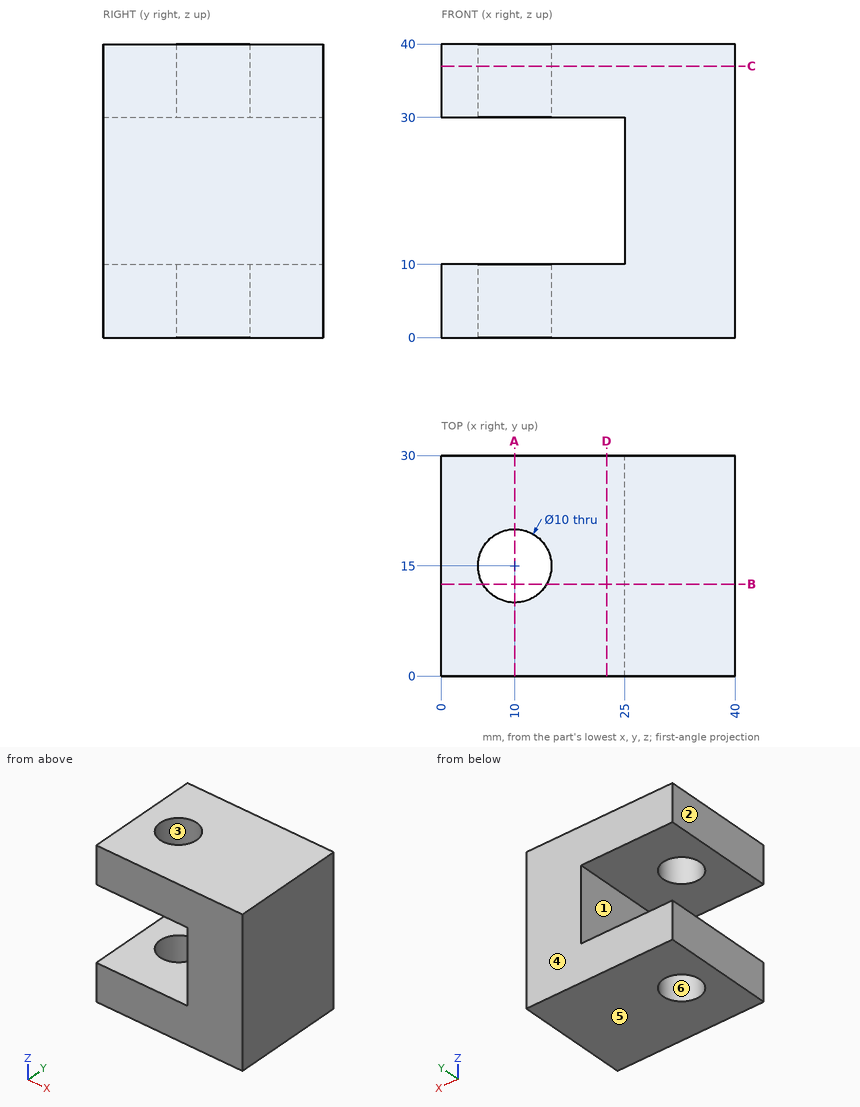
Drawing for the job (mm, zero at the part's lowest x, y, z). A direction names the side the tool comes from. Give positions to 0.01 mm unless a question says otherwise; leave off trailing zeros. Loops run counter-clockwise (first coordinate to the right, second up) from the corner with the lowest first, then second, coordinate; pieces in that order, holes last.
1) 3-axis set-ups, long thin cutter, end or side, ignore diameter. For the marked faces 1 and 2: which of +Z, -Z, +X, -X, +Y, -Y reach the whole face in a straight line?
Values follow:
face 1: -X, +Y, -Y
face 2: +Z, -Z, -X, +Y, -Y
2) Band-saw the part on A-A on x = 10. List the corners of the cut face in (y, z).
Values follow:
outline: (0, 0) - (10, 0) - (10, 10) - (0, 10) - close; (0, 30) - (10, 30) - (10, 40) - (0, 40) - close; (20, 0) - (30, 0) - (30, 10) - (20, 10) - close; (20, 30) - (30, 30) - (30, 40) - (20, 40) - close
3) Band-saw the part on B-B on y = 12.5. List the corners of the cut face in (x, z).
Values follow:
outline: (0, 0) - (5.67, 0) - (5.67, 10) - (0, 10) - close; (0, 30) - (5.67, 30) - (5.67, 40) - (0, 40) - close; (14.33, 0) - (40, 0) - (40, 40) - (14.33, 40) - (14.33, 30) - (25, 30) - (25, 10) - (14.33, 10) - close
4) Two-plate mould, pull along Y, no slides. Class the marked faces 3, 4, 5 and 6: released by +Y, released by -Y, zero draft, split by the parting line, or undercut.
Values follow:
face 3: undercut
face 4: released by +Y
face 5: zero draft
face 6: undercut
5) Band-saw the part on D-D on x = 22.5. List the corners of the cut face in (y, z), then the cut area to 3 significant figures.
Values follow:
outline: (0, 0) - (30, 0) - (30, 10) - (0, 10) - close; (0, 30) - (30, 30) - (30, 40) - (0, 40) - close
area: 600 mm2
6) Band-saw the part on C-C on z = 37. List the corners of the cut face in (x, y), then the cut area to 3 significant figures.
Values follow:
outline: (0, 0) - (40, 0) - (40, 30) - (0, 30) - close; hole circle Ø10 at (10, 15)
area: 1,120 mm2
7) Probe line 1 along Y through (x, z) = (10, 32.75); line 2 along Z through (x, y) = (19.5, 2.25); line 3 along X through (y, z) = (12.25, 12). List the from-to ranges inside material, lowest first.
Values follow:
line 1: y = 0 to 10, 20 to 30
line 2: z = 0 to 10, 30 to 40
line 3: x = 25 to 40
8) Drop flat-ended pins along their axis: P1, Ø9, axis at x = 10, y = 15, coming from the -Z side; P2, Ø8, axis at y = 14.5, z = 14.5, coming from the -X side. Give the stop position or say it passes through.
Values follow:
P1: passes through
P2: stops at x = 25
